Read the model definition and answer for the solid it produces. Units are mm, in the model's axes. A direction names the side the tool comes from. Coordinates: 2 decimals unless noted, no trailing zeros. Loops run counter-clockwise (first coordinate to the right, second up) from the corner with the lowest first, then second, coordinate; pieces in that order, holes last. Notation, with made-up numbers: (16, 21.5) -> (72, 21.5) arc R14 cw to (72, 43.5) -> close; hole circle Ø6 at (11, 22). An arc over 180 degrees is marked (long way). Answer in a Markdown table with one row per item.
```python
from build123d import *

# Parameters (mm, degrees)
SKETCH_1_W          = 8
SKETCH_1_H          = 8
SKETCH_1_W_2        = 6
SKETCH_1_H_2        = 6
EXTRUDE_1_DEPTH     = 55
SKETCH_3_R          = 1.55
CUT_EXTRUDE_1_DEPTH = 55


with BuildPart() as part:
    # 草图1 → 凸台-拉伸1 (new body)
    with BuildSketch(Plane.XY):
        Rectangle(SKETCH_1_W, SKETCH_1_H)
        Rectangle(SKETCH_1_W_2, SKETCH_1_H_2, mode=Mode.SUBTRACT)
    extrude(amount=-EXTRUDE_1_DEPTH)

    # 草图3 → 切除-拉伸1 (cut)
    with BuildSketch(Plane(origin=(0, 4, 0), x_dir=(1, 0, 0), z_dir=(0, 1, 0))):
        with Locations(Location((0, 3.5, 0), (0, 0, 90))):
            Circle(SKETCH_3_R)
        with Locations(Location((0, 11.5, 0), (0, 0, 90))):
            Circle(SKETCH_3_R)
        with Locations(Location((0, 43.5, 0), (0, 0, 90))):
            Circle(SKETCH_3_R)
        with Locations(Location((0, 51.5, 0), (0, 0, 90))):
            Circle(SKETCH_3_R)
    extrude(amount=-CUT_EXTRUDE_1_DEPTH, mode=Mode.SUBTRACT)


solid = part.part
```
1. A cutting plane is placed at A-A on y = 1.5. Give the vertices of the cut face in (x, z).
A:
| item | result |
|---|---|
| outline | (-4, -55) -> (-3, -55) -> (-3, 0) -> (-4, 0) -> close; (3, -55) -> (4, -55) -> (4, 0) -> (3, 0) -> close |
2. Find the intervals of material crossed by probe 1 along Y at (x, z) = (0, -15); probe 2 along X at (y, z) = (-3.65, -11.5), in increasing order.
A:
| item | result |
|---|---|
| probe 1 | y = -4 to -3, 3 to 4 |
| probe 2 | x = -4 to -1.55, 1.55 to 4 |
3. A cutting plane is placed at D-D on x = 0. Count the separate pieces of the cut face and the enclosed holes in it, and give its area (3 significant figures).
A:
| item | result |
|---|---|
| separate pieces | 10 |
| enclosed holes | 0 |
| area | 85.2 mm2 |
4. A cutting plane is placed at B-B on z = -43.5. Give the vertices of the cut face in (x, y).
A:
| item | result |
|---|---|
| outline | (-4, -4) -> (-1.55, -4) -> (-1.55, -3) -> (-3, -3) -> (-3, 3) -> (-1.55, 3) -> (-1.55, 4) -> (-4, 4) -> close; (1.55, -4) -> (4, -4) -> (4, 4) -> (1.55, 4) -> (1.55, 3) -> (3, 3) -> (3, -3) -> (1.55, -3) -> close |
5. The mould has two halves that part along X. Classify faces 3 (the flat face through (4, 0, -27)), 4 (the flat face through (0, -3, -27)), 5 (the cylindrical face through (-0.07, 3.51, -9.95)), 6 (the flat face through (0, -4, -27)): pulls with the +X half, pulls with the -X half, needs draft (parallel to the pull), parting line crosses it, or undercut.
A:
| item | result |
|---|---|
| face 3 | pulls with the +X half |
| face 4 | undercut |
| face 5 | undercut |
| face 6 | needs draft |
6. A tool of negligible diameter and unlimited length cuts with its end or side. For faces 1 (the flat face through (-3, 0, -27)), 2 (the cylindrical face through (-0.466, -3.493, -52.978)), from which of +Z, -Z, +X, -X, +Y, -Y can it reach the whole face along a straight path? Write none if from no direction.
A:
| item | result |
|---|---|
| face 1 | +Z, -Z |
| face 2 | +Y, -Y |
